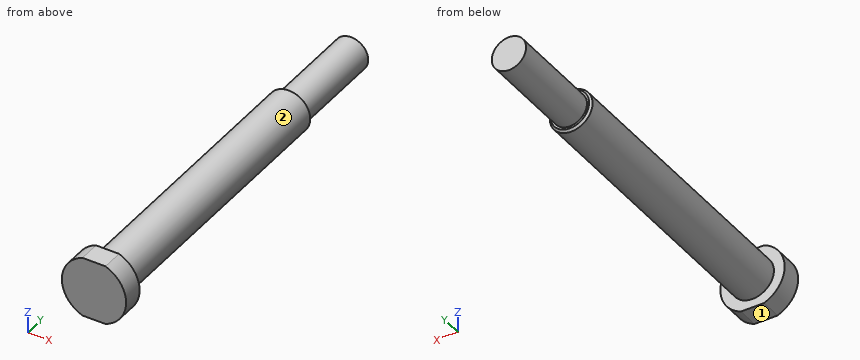
```python
from build123d import *

# Parameters (mm, degrees)
CHAMFER_1_SIZE      = 1
SKETCH_2_W          = 36.885897288
SKETCH_2_H          = 4.926272709
SKETCH_2_W_2        = 40.411275082
SKETCH_2_H_2        = 4.776597597
CUT_EXTRUDE_1_DEPTH = 30


with BuildPart() as part:
    # 草图1 → 旋转1 (revolve)
    with BuildSketch(Plane.XY, mode=Mode.PRIVATE) as revolve_1_sk:
        Polygon((0, 95), (0, -95), (15, -95), (15, -85), (10, -85), (10, 50), (8, 50), (8, 95), align=None)
    revolve(revolve_1_sk.sketch.rotate(Axis((0, 95, 0), (0, -1, 0)), 180), axis=Axis((0, 95, 0), (0, -1, 0)))

    # 倒角1
    chamfer_1_edges = [part.edges().sort_by_distance(p)[0] for p in [
        (10, 50, 0),
    ]]
    chamfer(chamfer_1_edges, length=CHAMFER_1_SIZE)

    # 草图2 → 切除-拉伸1 (cut)
    with BuildSketch(Plane(origin=(0, -85, 0), x_dir=(1, 0, 0), z_dir=(0, 1, 0))):
        with Locations((-1.52363424, -16.463136355)):
            Rectangle(SKETCH_2_W, SKETCH_2_H)
        with Locations((0.239054657, 16.388298799)):
            Rectangle(SKETCH_2_W_2, SKETCH_2_H_2)
    extrude(amount=-CUT_EXTRUDE_1_DEPTH, mode=Mode.SUBTRACT)


solid = part.part
```
Can you work these out from the model? Positions are in its coordinate system, mm. Face numbers are marked on the shaded views. A direction names the side the tool comes from. Coordinates: 2 decimals unless noted, no trailing zeros. Loops run counter-clockwise (first coordinate to the right, second up) from the corner with the lowest first, then second, coordinate; pieces in that order, holes last. Notation, with made-up numbers: (6, 43.25) -> (37, 43.25) arc R29 cw to (37, 71.25) -> close; hole circle Ø11 at (-17.75, 86.25). An arc over 180 degrees is marked (long way). Put each result on its own line as item: value. Start each with the question number.
Q1. I want a section at B-B (z = 0). Write out the boundary of the cut face in (x, y), plus the area to 3 significant figures.
Q2. I want a section at A-A (x = 0). Write out the boundary of the cut face in (y, z), plus the area to 3 significant figures.
Q3. I want a section at C-C (y = 64). Write out the boundary of the cut face in (x, z), plus the area to 3 significant figures.
Q4. I'm going to push flat-ended pins straight in: P1, Ø3, axis at y = 9, z = -6.5, coming from the +X side; P2, Ø1.5, axis at x = -5.5, y = 18, coming from the -Z side; P3, Ø2, axis at y = -13.5, z = -6.5, coming from the -X side. Where does each tip first touch, or does it pass through?
Q5. For the marked faces 1 and 2, which set-ups out of +Z, -Z, +X, -X, +Y, -Y let a thin tool reach every point of the face, with its end or its side?
Q6. I want a section at D-D (x = -12). Write out the boundary of the cut face in (y, z), plus the area to 3 significant figures.
Q7. If I drill on line 1 (Y direction, x = -1, z = 12.75); line 2 (Y direction, x = -1, z = 8.5); line 3 (X direction, y = -39.5, z = 8.75), over which ranges is the centre line in solid material (lowest first)? Write a range as [from, to].
Taken from the geometry:
1. outline: (-15, -95) -> (15, -95) -> (15, -85) -> (10, -85) -> (10, 49) -> (9, 50) -> (8, 50) -> (8, 95) -> (-8, 95) -> (-8, 50) -> (-9, 50) -> (-10, 49) -> (-10, -85) -> (-15, -85) -> close
1. area: 3,720 mm2
2. outline: (-95, -14) -> (-85, -14) -> (-85, -10) -> (49, -10) -> (50, -9) -> (50, -8) -> (95, -8) -> (95, 8) -> (50, 8) -> (50, 9) -> (49, 10) -> (-85, 10) -> (-85, 14) -> (-95, 14) -> close
2. area: 3,700 mm2
3. outline: circle Ø16 at (0, 0)
3. area: 201 mm2
4. P1: stops at x = 8.66
4. P2: stops at z = -8.8
4. P3: stops at x = -8.35
5. face 1: -Z, +X, -X, +Y, -Y
5. face 2: +Y
6. outline: (-95, -9) -> (-85, -9) -> (-85, 9) -> (-95, 9) -> close
6. area: 180 mm2
7. line 1: y = [-95, -85]
7. line 2: y = [-95, 50]
7. line 3: x = [-4.84, 4.84]
